Geometry: see drawing. Coordinates: mm, zero at the bounding-box minimum. A direction names the side the tool comes from. Coordinates: 2 decimals unless noted, no trailing zeros. Loops run counter-clockwise (first coordinate to the right, second up) from the corner with the lowest first, then second, coordinate; pieces in that order, holes last. Notation, with made-up numbers: M -9,68.25 L 11,68.25 A14 ccw 11,76.25 Z; hole C 8.5,46.25 d3. An arc over 180 degrees is marked long. One line per question, with ' | ' between items. Start each with the question number.
1. Access query for the marked faces 1, 2 and 3. Directions: +Z, -Z, +X, -X, +Y, -Y. A direction counts if a zero-diameter tool reaches every point of the face in a straight line with its end or side. Return the directions, or none.
2. Section query D-D, the plane z = 2.25. Output: boundary loops of the cut face in (x, y).
3. Section query B-B, the plane x = 4.5. Output: boundary loops of the cut face in (y, z) (1 decimal), and give its area (3 significant figures).
4. Pin query (flat end, axial travel): P1, Ø1.5, axis at y = 19.5, z = 10.5, coming from the +X side; P2, Ø1.5, axis at x = 10, y = 13.5, coming from the +Z side; P3, Ø5, axis at y = 25.5, z = 4, coming from the -X side. Return the tip coordinate at first contact, or that it passes through.
5. Section query A-A, the plane z = 8. Output: boundary loops of the cut face in (x, y), and give its area (3 significant figures).
6. Mould query, pull axis Z, two halves, no side actions, for the marked faces 4, 5 and 6. Classes: pulls with the +Z half, pulls with the -Z half, needs draft (parallel to the pull), parting line crosses it, or undercut.
7. Ray query, probe 1 along Y at (x, z) = (14.75, 10.5); probe 2 along Z at (x, y) = (5, 29.5) (1 decimal); probe 3 along X at (y, z) = (5.5, 7.75). Return the intervals inside material, ascending.
8. Section query C-C, the plane y = 15. Output: boundary loops of the cut face in (x, z).
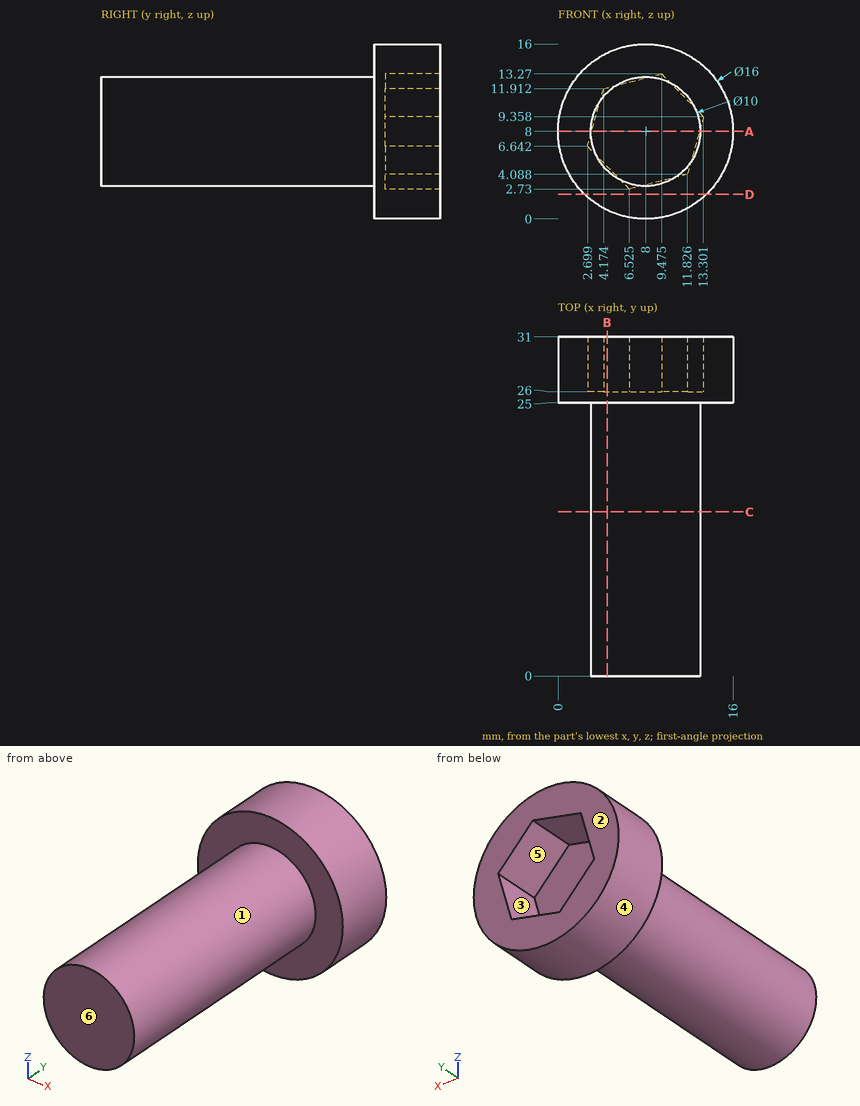
Taken from the geometry:
1) face 1: -Y | face 2: +Z, -Z, +X, -X, +Y | face 3: +Y
2) outline: M 2.44,25 L 13.56,25 L 13.56,31 L 2.44,31 Z
3) outline: M 0,4.4 L 25,4.4 L 25,0.8 L 31,0.8 L 31,4.8 L 26,4.8 L 26,12 L 31,12 L 31,15.2 L 25,15.2 L 25,11.6 L 0,11.6 Z | area: 229 mm^2
4) P1: x = 12.68 | P2: z = 12.84 | P3: x = 0.14
5) outline: M 0,25 L 3,25 L 3,0 L 13,0 L 13,25 L 16,25 L 16,31 L 12.92,31 L 12.92,26 L 3.08,26 L 3.08,31 L 0,31 Z | area: 297 mm^2
6) face 4: parting line crosses it | face 5: undercut | face 6: needs draft
7) probe 1: 25 to 31 | probe 2: 0.6 to 4.3, 12.1 to 15.4 | probe 3: 3.01 to 12.99
8) outline: C 8,8 d10
